The model under review builds one solid part; all positions refer to its coordinate system, in mm. A direction names the side the tool comes from. Round coordinates to 2 decimals unless told otherwise and drop trailing zeros. Write each loop counter-clockwise with the first axis right and the second up, starting at its lowest first coordinate (ties: lowest second). Pieces come first, ordered by that corner, then holes. Notation, with made-up numbers: (-10, 71) - (49, 71) arc R22 cw to (49, 84) - close; hole circle Ø7 at (-26, 56.5). An arc over 180 degrees is marked (long way). Return JSON: item names as keys, results as strings.
from build123d import *

# Parameters (mm, degrees)
SKETCH1_R           = 65
SKETCH1_R_2         = 2.5
BOSS_EXTRUDE1_DEPTH = 26
CUT_EXTRUDE1_DEPTH  = 96.530099969
SKETCH3_R           = 45
SKETCH3_R_2         = 15
CUT_EXTRUDE2_DEPTH  = 8
CUT_EXTRUDE3_START  = -8
SKETCH4_R           = 45
SKETCH4_R_2         = 15
CUT_EXTRUDE3_DEPTH  = 8


with BuildPart() as part:
    # Sketch1 → Boss-Extrude1 (new body)
    with BuildSketch(Plane.XY):
        with Locations(Location((0, 0, 0), (0, 0, 180))):
            Circle(SKETCH1_R)
        with Locations(Location((0, 55, 0), (0, 0, 180))):
            Circle(SKETCH1_R_2, mode=Mode.SUBTRACT)
        with Locations(Location((47.631397208, -27.5, 0), (0, 0, 180))):
            Circle(SKETCH1_R_2, mode=Mode.SUBTRACT)
        with Locations(Location((-47.631397208, -27.5, 0), (0, 0, 180))):
            Circle(SKETCH1_R_2, mode=Mode.SUBTRACT)
    extrude(amount=BOSS_EXTRUDE1_DEPTH)

    # Sketch2 → Cut-Extrude1 (cut, through all)
    with BuildSketch(Plane.XY.offset(26)):
        with BuildLine():
            Line((-1.5, 6.403418514), (1.5, 6.403418514))
            Line((1.5, 6.403418514), (1.5, 4.769696007))
            ThreePointArc((1.5, 4.769696007), (0, -5), (-1.5, 4.769696007))
            Line((-1.5, 4.769696007), (-1.5, 6.403418514))
        make_face()
    extrude(amount=-CUT_EXTRUDE1_DEPTH, mode=Mode.SUBTRACT)

    # Sketch3 → Cut-Extrude2 (cut)
    with BuildSketch(Plane.XY.offset(26)):
        Circle(SKETCH3_R)
        Circle(SKETCH3_R_2, mode=Mode.SUBTRACT)
    extrude(amount=-CUT_EXTRUDE2_DEPTH, mode=Mode.SUBTRACT)

    # Sketch4 → Cut-Extrude3 (cut)
    with BuildSketch(Plane(origin=(0, 0, 0), x_dir=(-1, 0, 0), z_dir=(0, 0, -1)).offset(CUT_EXTRUDE3_START)):
        with Locations(Location((0, 0, 0), (0, 0, 180))):
            Circle(SKETCH4_R)
        with Locations(Location((0, 0, 0), (0, 0, 180))):
            Circle(SKETCH4_R_2, mode=Mode.SUBTRACT)
    extrude(amount=CUT_EXTRUDE3_DEPTH, mode=Mode.SUBTRACT)


solid = part.part
(1) Clearance check with flat-ended pins moving along their axes: pin 1 Ø3.5 at (x, z) = (0.5, 7.5) entering from -Y; pin 2 Ø0.5 at (y, z) = (5.5, 13.5) entering from -X; pin 3 Ø8 at (x, y) = (-12.5, 35.5) entering from +Z; pin 4 Ø4 at (x, y) = (47.63, -27.5) entering from +Z. State where each tip first meets the part, or that it passes through.
Filled in:
{"pin 1": "stops at y = -65", "pin 2": "stops at x = -64.79", "pin 3": "stops at z = 18", "pin 4": "passes through"}
(2) Add section D-D (x = -48). Write out the cut boundary in (y, z).
Filled in:
{"outline": "(-43.83, 0) - (-29.97, 0) - (-29.97, 26) - (-43.83, 26) - close; (-25.03, 0) - (43.83, 0) - (43.83, 26) - (-25.03, 26) - close"}
(3) Mouldability with a two-part tool opening along X and no side actions: class faces 5 (the cylindrical face through (-62, -19.52, 12.82)), 6 (the flat face through (-14, -44, 26)), 7 (the cylindrical face through (-14.985, 0.66, 22.056)) as released by +X, released by -X, zero draft, split by the parting line, or undercut.
Filled in:
{"face 5": "split by the parting line", "face 6": "zero draft", "face 7": "undercut"}
(4) Add section A-A (z = 10). Write out the cut boundary in (x, y).
Filled in:
{"outline": "circle Ø130 at (0, 0); hole circle Ø5 at (-47.63, -27.5); hole circle Ø5 at (0, 55); hole (-1.5, 4.77) arc R5 ccw (long way) to (1.5, 4.77) - (1.5, 6.4) - (-1.5, 6.4) - close; hole circle Ø5 at (47.63, -27.5)"}
(5) Add section C-C (x = 0). Write out the cut boundary in (y, z).
Filled in:
{"outline": "(-65, 0) - (-45, 0) - (-45, 8) - (-15, 8) - (-15, 0) - (-5, 0) - (-5, 26) - (-15, 26) - (-15, 18) - (-45, 18) - (-45, 26) - (-65, 26) - close; (6.4, 0) - (15, 0) - (15, 8) - (45, 8) - (45, 0) - (52.5, 0) - (52.5, 26) - (45, 26) - (45, 18) - (15, 18) - (15, 26) - (6.4, 26) - close; (57.5, 0) - (65, 0) - (65, 26) - (57.5, 26) - close"}
(6) Wall thickness on line 1 (Y direction, x = 0, z = 17.5); line 2 (X direction, y = -10, z = 4.75); line 3 (Y direction, x = 7, z = 19.25): over which ranges is each line inside the solid? List them lowest first.
Filled in:
{"line 1": "y = -65 to -5, 6.4 to 52.5, 57.5 to 65", "line 2": "x = -64.23 to -43.87, -11.18 to 11.18, 43.87 to 64.23", "line 3": "y = -64.62 to -44.45, -13.27 to 13.27, 44.45 to 64.62"}
(7) For faces 1 (the flat face through (4, -4, 26)), 2 (the flat face through (0, 6.403, 13)), 3 (the cylindrical face through (20.765, -39.923, 22.056)), 4 (the cylindrical face through (8.06, -12.65, 4.06)), list the 3-axis set-ups (+Z, -Z, +X, -X, +Y, -Y) from which the entire face can be reached by the end or side of a thin tool; tool diameter is ignored.
Filled in:
{"face 1": "+Z, +X, -X, +Y, -Y", "face 2": "+Z, -Z", "face 3": "+Z", "face 4": "-Z"}
(8) Add section B-B (y = 0). Write out the cut boundary in (x, z), plus the area to 3 significant figures.
Filled in:
{"outline": "(-65, 0) - (-45, 0) - (-45, 8) - (-15, 8) - (-15, 0) - (-5, 0) - (-5, 26) - (-15, 26) - (-15, 18) - (-45, 18) - (-45, 26) - (-65, 26) - close; (5, 0) - (15, 0) - (15, 8) - (45, 8) - (45, 0) - (65, 0) - (65, 26) - (45, 26) - (45, 18) - (15, 18) - (15, 26) - (5, 26) - close", "area": "2,160 mm2"}
